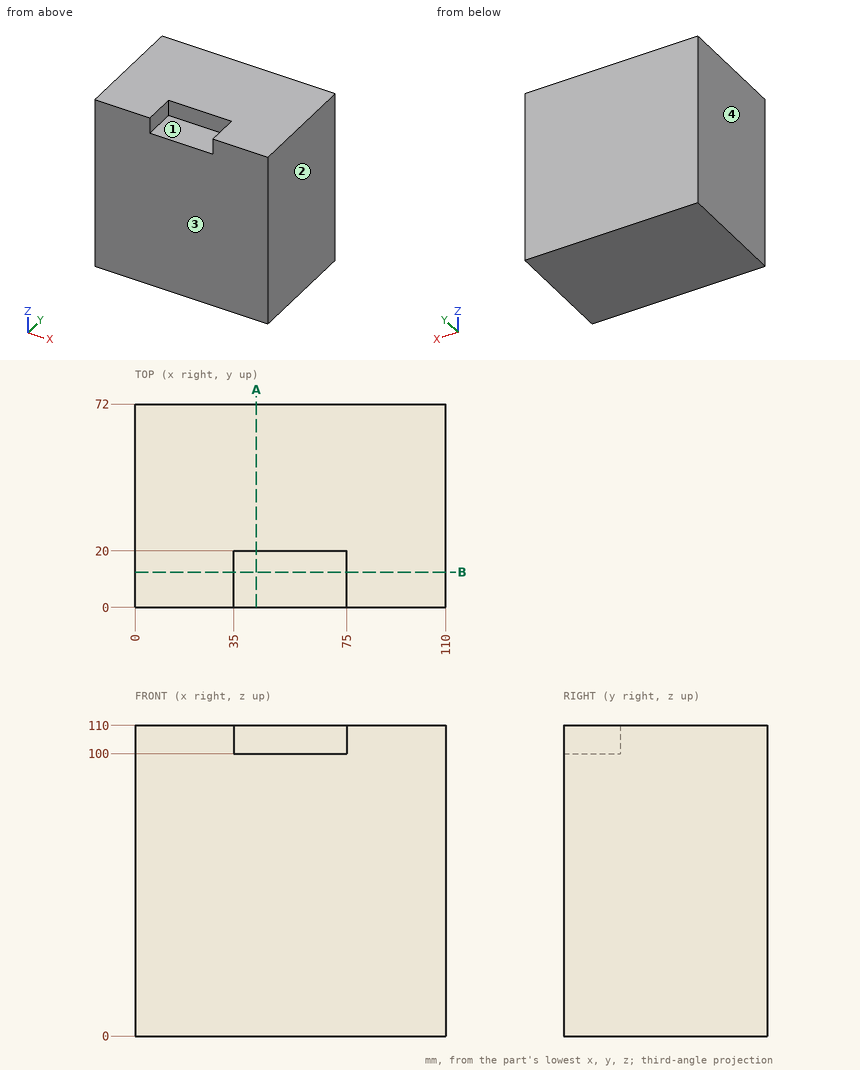
Here's the drawing with two shaded views (mm, measured from the low corner). I have some questions. Round coordinates to 2 decimals unless told otherwise and drop trailing zeros. Write each loop counter-clockwise with the first axis right and the second up, starting at its lowest first coordinate (ties: lowest second). Pieces come first, ordered by that corner, then holes.
(1) If I drill on probe 1 along X at (y, z) = (9.5, 102.5), over which ranges is the centre line in solid material (lowest first)?
Findings below:
probe 1: x = 0 to 35, 75 to 110
(2) Suppose I cut it at A-A on x = 43. Write out the boundary of the cut face in (y, z), and give its area (3 significant figures).
Findings below:
outline: (0, 0) - (72, 0) - (72, 110) - (20, 110) - (20, 100) - (0, 100) - close
area: 7,720 mm2
(3) Suppose I cut it at B-B on y = 12.5. Write out the boundary of the cut face in (x, z), and give its area (3 significant figures).
Findings below:
outline: (0, 0) - (110, 0) - (110, 110) - (75, 110) - (75, 100) - (35, 100) - (35, 110) - (0, 110) - close
area: 11,700 mm2
(4) Thinking about a two-plate mould opening in X: for the marked faces 1, 2, 3 and 4, which applies, +X half, -X half, draft (parallel to the pull), parting line (faces both ways), or undercut?
Findings below:
face 1: undercut
face 2: +X half
face 3: draft
face 4: -X half
